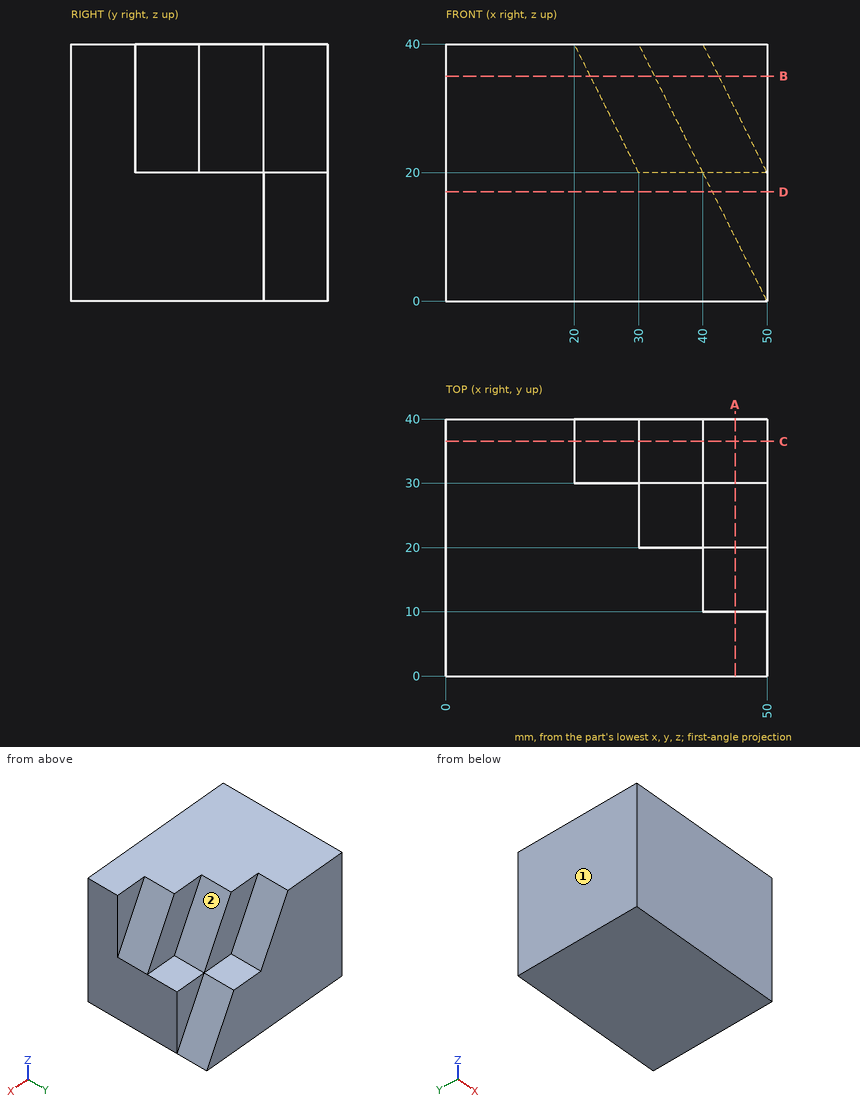
Geometry: see drawing. Coordinates: mm, zero at the bounding-box minimum. A direction names the side the tool comes from. Coordinates: 2 decimals unless noted, no trailing zeros. Loops run counter-clockwise (first coordinate to the right, second up) from the corner with the lowest first, then second, coordinate; pieces in that order, holes last.
(1) Material intervals for probe 1 along Z at (x, y) = (35, 31); probe 2 along Y at (x, z) = (29, 31.5); probe 3 along X at (y, z) = (32, 14), sorted ascending.
(2) First-contact query: pin 1 Ø8 at (x, z) = (46.5, 27.5) entering from +Y; pin 2 Ø5 at (x, y) = (33.5, 33.5) entering from +Z; pin 3 Ø11 at (x, y) = (44.5, 26) entering from +Z. Flat tips, straight axial feed; report the tip coordinate or a pass-through.
(3) Section A-A on x = 45. Return the cut outline in (y, z), then the cut area to 3 significant figures.
(4) Set-up query: the marked faces 1 and 2. Return all of +Z, -Z, +X, -X, +Y, -Y with unobstructed straight access to the full face (end or side cutting, diameter ignored); none if empty.
(5) Section C-C on y = 36.5. Return the cut outline in (x, z), then the cut area to 3 significant figures.
(6) Section B-B on z = 35. Return the cut outline in (x, y).
(7) Section D-D on z = 17. Return the cut outline in (x, y), then the cut area to 4 significant figures.
Data:
1. probe 1: z = 0 to 20
1. probe 2: y = 0 to 30
1. probe 3: x = 0 to 43
2. pin 1: stops at y = 20
2. pin 2: stops at z = 20
2. pin 3: stops at z = 22
3. outline: (0, 0) - (40, 0) - (40, 10) - (30, 10) - (30, 20) - (20, 20) - (20, 30) - (10, 30) - (10, 40) - (0, 40) - close
3. area: 1,000 mm2
4. face 1: +Z, -Z, -X, +Y, -Y
4. face 2: +Z, +X, +Y
5. outline: (0, 0) - (50, 0) - (40, 20) - (30, 20) - (20, 40) - (0, 40) - close
5. area: 1,400 mm2
6. outline: (0, 0) - (50, 0) - (50, 10) - (42.5, 10) - (42.5, 20) - (32.5, 20) - (32.5, 30) - (22.5, 30) - (22.5, 40) - (0, 40) - close
7. outline: (0, 0) - (50, 0) - (50, 30) - (41.5, 30) - (41.5, 40) - (0, 40) - close
7. area: 1,915 mm2
